from build123d import *

# Parameters (mm, degrees)
SKETCH1_W                      = 46
SKETCH1_H                      = 55
BOSS_EXTRUDE1_DEPTH            = 20
CUT_EXTRUDE1_DEPTH             = 58.203583804
SKETCH3_R                      = 6.75
CUT_EXTRUDE2_DEPTH             = 47.296696276
SKETCH4_R                      = 2.5
CUT_EXTRUDE3_DEPTH             = 54.714523176
SKETCH6_W                      = 8
SKETCH6_H                      = 37
CUT_EXTRUDE4_DEPTH             = 54.714523176
CUT_EXTRUDE5_DEPTH             = 16
CUT_EXTRUDE6_DEPTH             = 58.203583804
SKETCH9_R                      = 8
CUT_EXTRUDE7_DEPTH             = 7
CHAMFER1_SIZE                  = 2
F_5_5_5_5_DIAMETER_HOLE1_D     = 5.5
SKETCH12_R                     = 4.75
CUT_EXTRUDE8_DEPTH             = 42.723313638
M3_TAPPED_HOLE2_D              = 2.5
M3_TAPPED_HOLE2_DEPTH          = 7.5
M3_TAPPED_HOLE2_TIP            = 0.751075774
SKETCH17_W                     = 0.5
SKETCH17_H                     = 27.5
CUT_EXTRUDE9_DEPTH             = 46.088447741
SKETCH18_W                     = 7.5
SKETCH18_H                     = 10
CUT_EXTRUDE10_DEPTH            = 46.088447741
F_4_5_4_5_DIAMETER_HOLE1_D     = 4.5
F_4_5_4_5_DIAMETER_HOLE1_DEPTH = 7.25
M4_TAPPED_HOLE1_D              = 3.3
M4_TAPPED_HOLE2_D              = 3.3
M4_TAPPED_HOLE2_DEPTH          = 10.1
M4_TAPPED_HOLE2_TIP            = 0.991420021
CHAMFER3_SIZE                  = 5
CHAMFER4_SIZE                  = 0.3
CUT_EXTRUDE11_DEPTH            = 46.088447741


with BuildPart() as part:
    # Sketch1 → Boss-Extrude1 (new, symmetric)
    with BuildSketch(Plane.XY):
        Rectangle(SKETCH1_W, SKETCH1_H)
    extrude(amount=BOSS_EXTRUDE1_DEPTH, both=True)

    # Sketch2 → Cut-Extrude1 (cut, through all)
    with BuildSketch(Plane(origin=(23, 0, 0), x_dir=(0, 0, -1), z_dir=(1, 0, 0))):
        Polygon((-12, 27.5), (20, 27.5), (20, -9.5), (-7.128857589, -9.5), align=None)
    extrude(amount=-CUT_EXTRUDE1_DEPTH, mode=Mode.SUBTRACT)

    # Sketch3 → Cut-Extrude2 (cut, through all)
    with BuildSketch(Plane(origin=(0, -1.084394382, 8.236793088), x_dir=(-1, 0, 0), z_dir=(0, 0.13052619222004844, -0.9914448613738109))):
        with Locations(Location((0, 2.331047994, 0), (0, 0, 90))):
            Circle(SKETCH3_R)
    extrude(amount=-CUT_EXTRUDE2_DEPTH, mode=Mode.SUBTRACT)

    # Sketch4 → Cut-Extrude3 (cut, through all)
    with BuildSketch(Plane.XY.offset(20)):
        with Locations((0, -18)):
            Circle(SKETCH4_R)
    extrude(amount=-CUT_EXTRUDE3_DEPTH, mode=Mode.SUBTRACT)

    # Sketch6 → Cut-Extrude4 (cut, through all)
    with BuildSketch(Plane(origin=(0, 0, -20), x_dir=(-1, 0, 0), z_dir=(0, 0, -1))):
        with Locations((-19, 9)):
            Rectangle(SKETCH6_W, SKETCH6_H)
        with Locations((19, 9)):
            Rectangle(SKETCH6_W, SKETCH6_H)
    extrude(amount=-CUT_EXTRUDE4_DEPTH, mode=Mode.SUBTRACT)

    # Sketch7 → Cut-Extrude5 (cut, symmetric)
    with BuildSketch(Plane(origin=(0, 0, 0), x_dir=(0, 0, -1), z_dir=(1, 0, 0))):
        Polygon((-7.128857589, -9.5), (20, -9.5), (20, -27.5), (-4.759112633, -27.5), align=None)
    extrude(amount=CUT_EXTRUDE5_DEPTH, both=True, mode=Mode.SUBTRACT)

    # Sketch8 → Cut-Extrude6 (cut, through all)
    with BuildSketch(Plane(origin=(23, 0, 0), x_dir=(0, 0, -1), z_dir=(1, 0, 0))):
        Polygon((4.974689938, -9.5), (7.344434894, -27.5), (20, -27.5), (20, -9.5), align=None)
    extrude(amount=-CUT_EXTRUDE6_DEPTH, mode=Mode.SUBTRACT)

    # Sketch9 → Cut-Extrude7 (cut)
    with BuildSketch(Plane(origin=(0, -1.084394382, 8.236793088), x_dir=(-1, 0, 0), z_dir=(0, 0.13052619222004838, -0.9914448613738109))):
        with Locations(Location((0, 2.331047994, 0), (0, 0, 90))):
            Circle(SKETCH9_R)
    extrude(amount=-CUT_EXTRUDE7_DEPTH, mode=Mode.SUBTRACT)

    # Chamfer1
    chamfer1_edges = [part.edges().sort_by_distance(p)[0] for p in [
        (15, 27.5, 16),
        (-15, 27.5, 16),
    ]]
    chamfer(chamfer1_edges, length=CHAMFER1_SIZE)

    # Ø5.5 (5.5) Diameter Hole1 (through all)
    with Locations(Plane.XY.offset(20)):
        with Locations((-10, -15.5), (10, -15.5)):
            Hole(F_5_5_5_5_DIAMETER_HOLE1_D / 2)

    # Sketch12 → Cut-Extrude8 (cut, through all)
    with BuildSketch(Plane.XY.offset(14)):
        with Locations((-10, -15.5)):
            Circle(SKETCH12_R)
        with Locations((10, -15.5)):
            Circle(SKETCH12_R)
    extrude(amount=-CUT_EXTRUDE8_DEPTH, mode=Mode.SUBTRACT)

    # M3 Tapped Hole2
    with Locations(Plane(origin=(0, -1.084394382, 8.236793088), x_dir=(-1, 0, 0), z_dir=(0, 0.13052619222004838, -0.9914448613738109))):
        with Locations((12, 25.831047994), (12, -23.168952006), (-12, -23.168952006)):
            Hole(M3_TAPPED_HOLE2_D / 2, depth=M3_TAPPED_HOLE2_DEPTH)
            with Locations((0, 0, -(M3_TAPPED_HOLE2_DEPTH + M3_TAPPED_HOLE2_TIP / 2))):  # 118° drill point
                Cone(0, M3_TAPPED_HOLE2_D / 2, M3_TAPPED_HOLE2_TIP, mode=Mode.SUBTRACT)

    # Sketch17 → Cut-Extrude9 (cut, through all)
    with BuildSketch(Plane.XY.offset(20)):
        with Locations((0, 13.75)):
            Rectangle(SKETCH17_W, SKETCH17_H)
    extrude(amount=-CUT_EXTRUDE9_DEPTH, mode=Mode.SUBTRACT)

    # Sketch18 → Cut-Extrude10 (cut, through all)
    with BuildSketch(Plane.XY.offset(20)):
        with Locations((-11.25, 15.5)):
            Rectangle(SKETCH18_W, SKETCH18_H)
        with Locations((11.25, 15.5)):
            Rectangle(SKETCH18_W, SKETCH18_H)
    extrude(amount=-CUT_EXTRUDE10_DEPTH, mode=Mode.SUBTRACT)

    # Ø4.5 (4.5) Diameter Hole1
    with Locations(Plane(origin=(7.5, 0, 0), x_dir=(0, 0, -1), z_dir=(1, 0, 0))):
        with Locations((-15.5, 15.5)):
            Hole(F_4_5_4_5_DIAMETER_HOLE1_D / 2, depth=F_4_5_4_5_DIAMETER_HOLE1_DEPTH)

    # M4 Tapped Hole1 (through all)
    with Locations(Plane.ZY.offset(7.5)):
        with Locations((15.5, 15.5)):
            Hole(M4_TAPPED_HOLE1_D / 2)

    # M4 Tapped Hole2
    with Locations(Plane(origin=(0, 0.481919925, -3.660545249), x_dir=(-1, 0, 0), z_dir=(0, 0.13052619222004835, -0.9914448613738109))):
        with Locations((-19, -13.723374809), (-19, -23.723374809), (19, -23.723374809), (19, -13.723374809)):
            Hole(M4_TAPPED_HOLE2_D / 2, depth=M4_TAPPED_HOLE2_DEPTH)
            with Locations((0, 0, -(M4_TAPPED_HOLE2_DEPTH + M4_TAPPED_HOLE2_TIP / 2))):  # 118° drill point
                Cone(0, M4_TAPPED_HOLE2_D / 2, M4_TAPPED_HOLE2_TIP, mode=Mode.SUBTRACT)

    # Chamfer3
    chamfer3_edges = [part.edges().sort_by_distance(p)[0] for p in [
        (-15, 10.5, 14.880953771),
        (15, 10.5, 14.880953771),
    ]]
    chamfer(chamfer3_edges, length=CHAMFER3_SIZE)

    # Chamfer4
    chamfer4_edges = [part.edges().sort_by_distance(p)[0] for p in [
        (0, -6.379224986, 14.600118138),
    ]]
    chamfer(chamfer4_edges, length=CHAMFER4_SIZE)

    # Sketch25 → Cut-Extrude11 (cut, through all)
    with BuildSketch(Plane.XY.offset(20)):
        with BuildLine():
            Line((2.5, -17.75), (2.5, -18.25))
            ThreePointArc((2.5, -18.25), (0, -20.75), (-2.5, -18.25))
            Line((-2.5, -18.25), (-2.5, -17.75))
            ThreePointArc((-2.5, -17.75), (0, -15.25), (2.5, -17.75))
        make_face()
    extrude(amount=-CUT_EXTRUDE11_DEPTH, mode=Mode.SUBTRACT)


solid = part.part
Design review of the part built by this model. Coordinates are the model's own, in mm. A direction names the side the tool comes from. Give positions to 0.01 mm unless a question says otherwise; leave off trailing zeros. Order: outer loops, then holes, each group sorted by start corner. A loop starts at its lowest first (then second) coordinate and runs counter-clockwise, first axis right, second up.
1. Add section B-B, the plane x = 1. State how many separate pieces and enclosed holes the cut face has, then the cut area to 3 significant figures.
Solution:
separate pieces: 3
enclosed holes: 1
area: 380 mm2
2. For pin 1 Ø5 at (x, y) = (9.5, -15) entering from -Z; pin 2 Ø3.5 at (y, z) = (15.5, 15.5) entering from +X; pin 3 Ø4 at (y, z) = (22, 14.5) entering from +X, all flat-tipped, find the tip position at first contact; note any pin that passes through.
Solution:
pin 1: stops at z = 14
pin 2: stops at x = -0.25
pin 3: stops at x = 15
3. Add section A-A, the plane y = 15.5. State the section outline as (x, z) points, then the cut area to 3 significant figures.
Solution:
outline: (-7.5, 10.42) - (-0.25, 10.42) - (-0.25, 13.85) - (-7.5, 13.85) - close; (-7.5, 17.15) - (-0.25, 17.15) - (-0.25, 20) - (-7.5, 20) - close; (0.25, 10.42) - (7.5, 10.42) - (7.5, 13.25) - (0.25, 13.25) - close; (0.25, 17.75) - (7.5, 17.75) - (7.5, 20) - (0.25, 20) - close
area: 82.4 mm2
4. Tool access review of faces 4 (the flat face through (-0.25, 17, 17)), 5 (the flat face through (-9, 10.5, 15)), 6 (the cylindrical face through (8.97, -20.137, 9.853)), 7 (the cylindrical face through (3.824, 13.504, 16.538)), 8 (the cylindrical face through (0.05, -20.75, 12.89)): name each direction out of +Z, -Z, +X, -X, +Y, -Y from which nothing blocks a thin tool from reaching the whole face with its end or side.
Solution:
face 4: +Z, -Z, +Y
face 5: +Z, -Z, -X
face 6: -Z
face 7: +X
face 8: +Z, -Z
5. Mouldability with a two-part tool opening along X and no side actions: class faces 1 (the flat face through (-15, -2, 13)), 2 (the flat face through (-19, -9.5, 7)), 3 (the conical face through (-11.97, -24.9, 13.29)) as +X half, -X half, draft (parallel to the pull), parting line (faces both ways), or undercut.
Solution:
face 1: -X half
face 2: draft
face 3: undercut
6. To check wall thickness, follow L1, parallel to X at y = 21, z = 16.25; L2, parallel to X at y = 15, z = 10.75; L3, parallel to X at y = -12, z = -3. State the ranges of each line that lie inside material, in increasing order.
Solution:
L1: x = -15 to -0.25, 0.25 to 15
L2: x = -7.5 to -0.25, 0.25 to 7.5
L3: x = -23 to -19.82, -18.18 to -16, 16 to 18.18, 19.82 to 23
